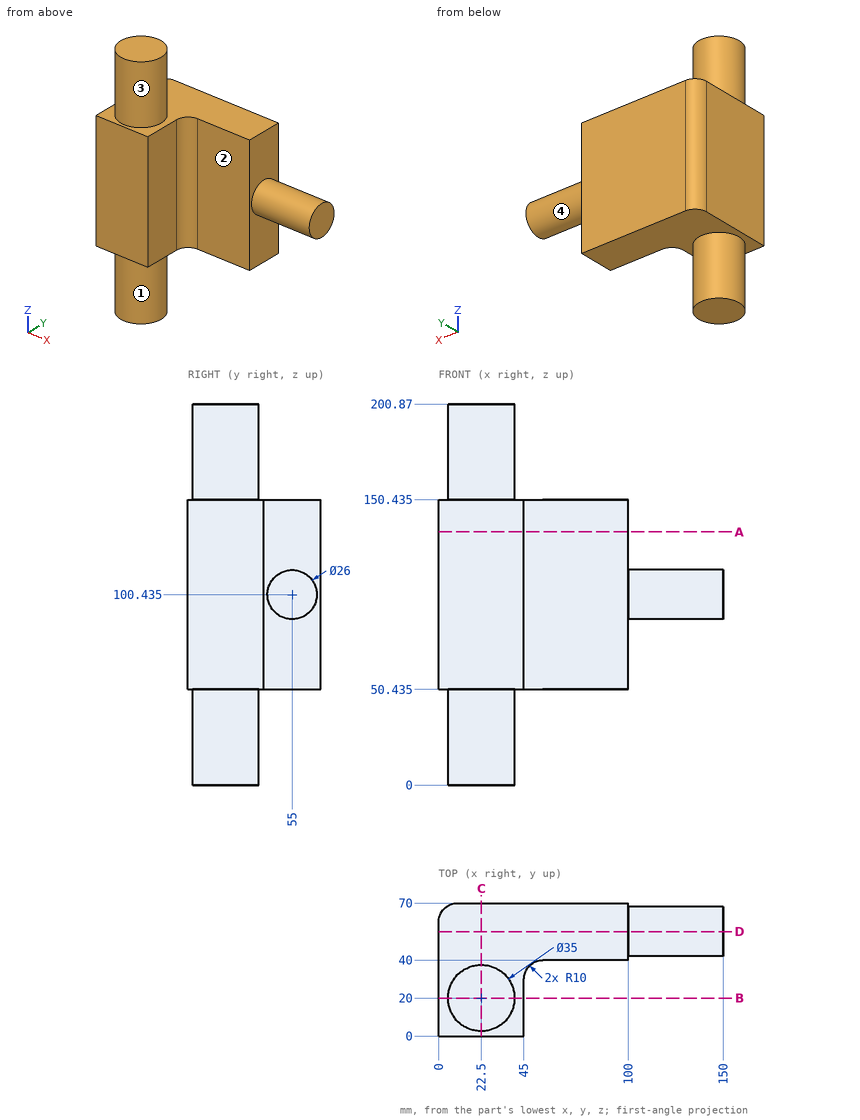
Check sheet for the drawn part. Datum: minimum x, y, z corner. Units: mm. A direction names the side the tool comes from. Round coordinates to 2 decimals unless told otherwise and drop trailing zeros. Write each loop counter-clockwise with the first axis right and the second up, starting at its lowest first coordinate (ties: lowest second). Pieces come first, ordered by that corner, then holes. Notation, with made-up numbers: (47.5, 55) -> (65.5, 55) arc R33 cw to (65.5, 87) -> close; hole circle Ø11 at (19, -5.5). An arc over 180 degrees is marked (long way). Put each result on its own line as item: value.
(1) Go/stop test with flat-tipped pins: pin 1 Ø6 at (x, y) = (90.5, 59.5) entering from +Z (3 decimals); pin 2 Ø13.5 at (x, z) = (87.5, 90) entering from -Y; pin 3 Ø8 at (x, y) = (112.5, 56.5) entering from +Z (3 decimals). Record where each tip stops, or that it passes through.
Values found:
pin 1: stops at z = 150.435
pin 2: stops at y = 40
pin 3: stops at z = 113.435
(2) Tool access check on the marked faces 1, 2, 3 and 4. Record the directions out of +Z, -Z, +X, -X, +Y, -Y that give a thin tool (end or side, any length) a straight path to the whole face; none if there is none.
Values found:
face 1: -Z
face 2: +Z, -Z, +X, -Y
face 3: +Z
face 4: +X
(3) Sectioned sample at A-A (z = 133.5). Enter the section's corners in (x, y), plus the area to 3 significant figures.
Values found:
outline: (0, 0) -> (45, 0) -> (45, 30) arc R10 cw to (55, 40) -> (100, 40) -> (100, 70) -> (10, 70) arc R10 ccw to (0, 60) -> close
area: 4,800 mm^2
(4) Sectioned sample at C-C (x = 22.5). Enter the section's corners in (y, z) (3 decimals).
Values found:
outline: (0, 50.435) -> (2.5, 50.435) -> (2.5, 0) -> (37.5, 0) -> (37.5, 50.435) -> (70, 50.435) -> (70, 150.435) -> (37.5, 150.435) -> (37.5, 200.87) -> (2.5, 200.87) -> (2.5, 150.435) -> (0, 150.435) -> close
(5) Sectioned sample at D-D (y = 55). Enter the section's corners in (x, z) (3 decimals), plus the area to 3 significant figures.
Values found:
outline: (0, 50.435) -> (100, 50.435) -> (100, 87.435) -> (150, 87.435) -> (150, 113.435) -> (100, 113.435) -> (100, 150.435) -> (0, 150.435) -> close
area: 11,300 mm^2
(6) Sectioned sample at B-B (y = 20). Enter the section's corners in (x, z) (3 decimals).
Values found:
outline: (0, 50.435) -> (5, 50.435) -> (5, 0) -> (40, 0) -> (40, 50.435) -> (45, 50.435) -> (45, 150.435) -> (40, 150.435) -> (40, 200.87) -> (5, 200.87) -> (5, 150.435) -> (0, 150.435) -> close
(7) Material ranges on line 1 (Z direction, x = 63.5, y = 45) (3 decimals); line 2 (X direction, y = 54, z = 83); line 3 (Y direction, x = 70.5, z = 99), recorded low to high.
Values found:
line 1: z = 50.435 to 150.435
line 2: x = 0 to 100
line 3: y = 40 to 70
